from build123d import *

# Parameters (mm, degrees)
SKETCH_1_W             = 15
SKETCH_1_H             = 15
EXTRUDE_1_DEPTH        = 90
SKETCH_2_R             = 3
CUT_EXTRUDE_1_DEPTH    = 4.5
SKETCH_3_R             = 2
CUT_EXTRUDE_2_DEPTH    = 92.549167118
PATTERN_LINEAR_1_COUNT = 4
PATTERN_LINEAR_1_PITCH = 60


with BuildPart() as part:
    # 草图1 → 凸台-拉伸1 (new, symmetric)
    with BuildSketch(Plane.XY):
        Rectangle(SKETCH_1_W, SKETCH_1_H)
    extrude(amount=EXTRUDE_1_DEPTH, both=True)

    # 草图2 → 切除-拉伸1 (cut)
    with BuildSketch(Plane(origin=(0, 7.5, 0), x_dir=(1, 0, 0), z_dir=(0, 1, 0))):
        with Locations(Location((0, -60, 0), (0, 0, 270))):
            Circle(SKETCH_2_R)
    cut_extrude_1 = extrude(amount=-CUT_EXTRUDE_1_DEPTH, mode=Mode.SUBTRACT)

    # 草图3 → 切除-拉伸2 (cut, through all)
    with BuildSketch(Plane(origin=(0, 7.5, 0), x_dir=(1, 0, 0), z_dir=(0, 1, 0))):
        with Locations(Location((0, -60, 0), (0, 0, 270))):
            Circle(SKETCH_3_R)
    cut_extrude_2 = extrude(amount=-CUT_EXTRUDE_2_DEPTH, mode=Mode.SUBTRACT)

    # 阵列(线性)1: 切除-拉伸1, 切除-拉伸2 ×4
    with Locations(*[(0, 0, -i * PATTERN_LINEAR_1_PITCH) for i in range(1, PATTERN_LINEAR_1_COUNT)]):
        add(cut_extrude_1, mode=Mode.SUBTRACT)
        add(cut_extrude_2, mode=Mode.SUBTRACT)


solid = part.part
CAD build for the part. Positions are in the model's coordinates, mm. A direction names the side the tool comes from. Coordinates: 2 decimals unless noted, no trailing zeros. Write each loop counter-clockwise with the first axis right and the second up, starting at its lowest first coordinate (ties: lowest second). Pieces come first, ordered by that corner, then holes. Notation, with made-up numbers: (61.5, 74.5) - (101.5, 74.5) arc R30 cw to (101.5, 108.5) - close; hole circle Ø3 at (65.25, 27.5). An arc over 180 degrees is marked (long way). Use a Markdown table: item, result. Add a question column.
Item 1: 3-axis set-ups, long thin cutter, end or side, ignore diameter. For faces 4 (the face through (0, 5, 57)), 5 (the face through (0, 0, 90)): which of +Z, -Z, +X, -X, +Y, -Y reach the whole face in a straight line?
Item 2: Drill centre lines: L1, parallel to Z at x = 0.75, y = -1.5; L2, parallel to X at y = 6.15, z = -60; L3, parallel to X at y = -4.75, z = -60. Where is each one in solid material? Low to high. Write a range as from..to.
Item 3: Band-saw the part on C-C, the plane y = 4.75. Give the cut face in (x, z), and give its area (3 significant figures).
Item 4: Band-saw the part on A-A, the plane z = 60. Give the cut face in (x, y).
Item 5: Flat gauge pins, fed straight in: pin 1 (8 mm diameter, centred on x = 0, z = -60, fed in from -Y); pin 2 (1.8 mm diameter, centred on x = 0.5, z = 58.5, fed in from +Y). Where does each tip first touch, or does it go through?
Item 6: Band-saw the part on B-B, the plane x = 0. Give the cut face in (y, z).
Item 7: Mould opens along X. For faces 1 (the face through (-0.766, -2.177, 1.847)), 2 (the face through (-3, 7.5, 1)), 3 (the face through (-7.5, 0, 1)) say: pulls with the +X half, pulls with the -X half, needs draft (parallel to the pull), parting line crosses it, or undercut.
Numbers:
| question | item | result |
|---|---|---|
| 1 | face 4 | +Y |
| 1 | face 5 | +Z, +X, -X, +Y, -Y |
| 2 | L1 | -90..-61.85, -58.15..-1.85, 1.85..58.15, 61.85..90 |
| 2 | L2 | -7.5..-3, 3..7.5 |
| 2 | L3 | -7.5..-2, 2..7.5 |
| 3 | outline | (-7.5, -90) - (7.5, -90) - (7.5, 90) - (-7.5, 90) - close; hole circle Ø6 at (0, -60); hole circle Ø6 at (0, 0); hole circle Ø6 at (0, 60) |
| 3 | area | 2,620 mm2 |
| 4 | outline | (-7.5, -7.5) - (-2, -7.5) - (-2, 3) - (-3, 3) - (-3, 7.5) - (-7.5, 7.5) - close; (2, -7.5) - (7.5, -7.5) - (7.5, 7.5) - (3, 7.5) - (3, 3) - (2, 3) - close |
| 5 | pin 1 | y = -7.5 |
| 5 | pin 2 | y = 3 |
| 6 | outline | (-7.5, -90) - (7.5, -90) - (7.5, -63) - (3, -63) - (3, -62) - (-7.5, -62) - close; (-7.5, -58) - (3, -58) - (3, -57) - (7.5, -57) - (7.5, -3) - (3, -3) - (3, -2) - (-7.5, -2) - close; (-7.5, 2) - (3, 2) - (3, 3) - (7.5, 3) - (7.5, 57) - (3, 57) - (3, 58) - (-7.5, 58) - close; (-7.5, 62) - (3, 62) - (3, 63) - (7.5, 63) - (7.5, 90) - (-7.5, 90) - close |
| 7 | face 1 | undercut |
| 7 | face 2 | needs draft |
| 7 | face 3 | pulls with the -X half |
